Work out the finished part from the listing and answer in its coordinate system (mm). Face numbers are marked on the shaded views. A direction names the side the tool comes from. Round coordinates to 2 decimals unless told otherwise and drop trailing zeros. Write each loop counter-clockwise with the first axis right and the second up, starting at its lowest first coordinate (ties: lowest second). Pieces come first, ordered by that corner, then holes. Notation, with made-up numbers: (-18, 64.25) - (39, 64.25) arc R14 cw to (39, 86.25) - close; hole circle Ø8 at (-39.5, -25.5). An arc over 180 degrees is marked (long way). Answer as a JSON object with one key per item and string values.
```python
from build123d import *


with BuildPart() as part:
    # Model → Revolve1 (revolve)
    with BuildSketch(Plane.XY, mode=Mode.PRIVATE) as revolve1_sk:
        Polygon((-193.071714982, -28.205353865), (-193.071714982, -27.205353865), (-170.52661738, -27.205353865), (-170.52661738, -26.205353865), (-99.022420086, -26.205353865), (-99.022420086, -27.205353865), (-53.071714982, -27.205353865), (-53.071714982, -28.205353865), (-41.671714982, -28.205353865), (-40.394954521, -28.205353865), (-39.894954521, -28.705353865), (-39.894954521, -31.205353865), (-206.248475443, -31.205353865), (-206.248475443, -28.705353865), (-205.748475443, -28.205353865), (-199.071714982, -28.205353865), align=None)
    revolve(revolve1_sk.sketch.rotate(Axis((-206.248475443, -31.205353865, 0), (-1, 0, 0)), 90), axis=Axis((-206.248475443, -31.205353865, 0), (-1, 0, 0)))


solid = part.part
```
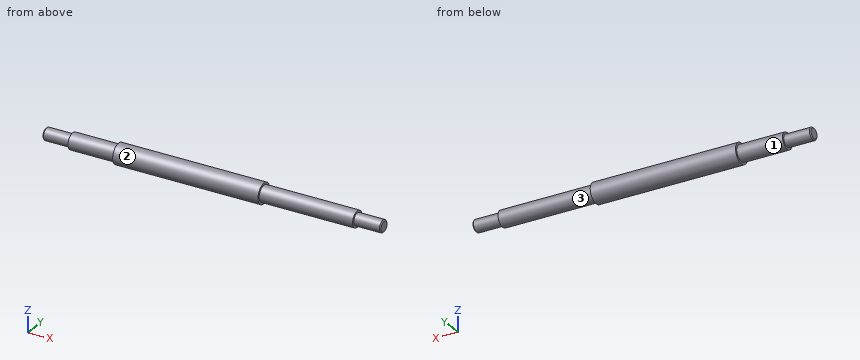
Item 1: Consider line 1 along X through (y, z) = (-33.5, -3.75); line 2 along Y through (x, z) = (-58.5, -0.5); line 3 along Y through (x, z) = (-138, -0.5). Determine where each line is inside the solid, lowest interval first.
Results found:
{"line 1": "-170.53 to -99.02", "line 2": "-35.17 to -27.24", "line 3": "-36.18 to -26.23"}
Item 2: Each of these flat-tipped pins is pushed along its axis until it touches: P1, Ø1, axis at x = -119.5, y = -27.5, coming from the +Z side; P2, Ø4, axis at x = -169, z = -3.5, coming from the +Y side; P3, Ø1, axis at x = -128, y = -28.5, coming from the -Z side. Where does it stop, or does it pass through?
Results found:
{"P1": "z = 3.84", "P2": "y = -26.44", "P3": "z = -4.49"}
Item 3: For the marked faces 1, 2 and 3, determine the directions among +Z, -Z, +X, -X, +Y, -Y from which every point of the face is accessible in a straight line to the end or side of a thin tool.
Results found:
{"face 1": "-X", "face 2": "+X, -X", "face 3": "+X"}
Item 4: A cutting plane is placed at B-B (x = -118). Write down the section's boundary in (y, z), and give its area (3 significant figures).
Results found:
{"outline": "circle Ø10 at (-31.21, 0)", "area": "78.5 mm²"}
Item 5: A cutting plane is placed at C-C (x = -50.5). Write down the section's boundary in (y, z).
Results found:
{"outline": "circle Ø6 at (-31.21, 0)"}
Item 6: A cutting plane is placed at A-A (z = 0). Write down the section's boundary in (x, y).
Results found:
{"outline": "(-206.25, -33.71) - (-205.75, -34.21) - (-193.07, -34.21) - (-193.07, -35.21) - (-170.53, -35.21) - (-170.53, -36.21) - (-99.02, -36.21) - (-99.02, -35.21) - (-53.07, -35.21) - (-53.07, -34.21) - (-40.39, -34.21) - (-39.89, -33.71) - (-39.89, -28.71) - (-40.39, -28.21) - (-53.07, -28.21) - (-53.07, -27.21) - (-99.02, -27.21) - (-99.02, -26.21) - (-170.53, -26.21) - (-170.53, -27.21) - (-193.07, -27.21) - (-193.07, -28.21) - (-205.75, -28.21) - (-206.25, -28.71) - close"}
